Here's how the part is built. I have some questions about the finished solid (model axes, mm). Face numbers are marked on the shaded views. A direction names the side the tool comes from. Give positions to 0.01 mm unless a question says otherwise; leave off trailing zeros. Loops run counter-clockwise (first coordinate to the right, second up) from the corner with the lowest first, then second, coordinate; pieces in that order, holes last.
Q1. I'm going to push flat-ended pins straight in: P1, Ø3, axis at x = -12, z = 16.5, coming from the +Y side; P2, Ø2, axis at x = -15, z = 17.5, coming from the -Y side; P3, Ø3, axis at x = -0.5, z = 9, coming from the +Y side; P4, Ø1, axis at x = 6, z = 11, coming from the +Y side. Where does each tip first touch, or does it pass through?
Q2. I need wall thicknesses on probe 1 along X at (y, z) = (-12.5, 17.75); probe 2 along X at (y, z) = (-7.5, 9.5); probe 3 along X at (y, z) = (-13, 8). Which ranges of each line are inside material? Lowest first, please.
Q3. Thinking about a two-plate mould opening in Z: for the marked faces 4, 5 and 6, which applies, pulls with the +Z half, pulls with the -Z half, needs draft (parallel to the pull), parting line crosses it, or undercut?
Q4. Suppose I cut it at B-B (x = -16). List the corners of the cut face in (y, z) for me.
Q5. Suppose I cut it at A-A (y = -7.5). List the corners of the cut face in (x, z) for me, and give its area (3 significant figures).
Q6. Suppose I cut it at C-C (y = -13.25). List the corners of the cut face in (x, z) for me.
Q7. Suppose I cut it at D-D (z = 13.25). List the corners of the cut face in (x, y) for me, and give its area (3 significant figures).
Q8. For the marked faces 1, 2 and 3, which set-ups out of +Z, -Z, +X, -X, +Y, -Y let a thin tool reach every point of the face, with its end or its side?
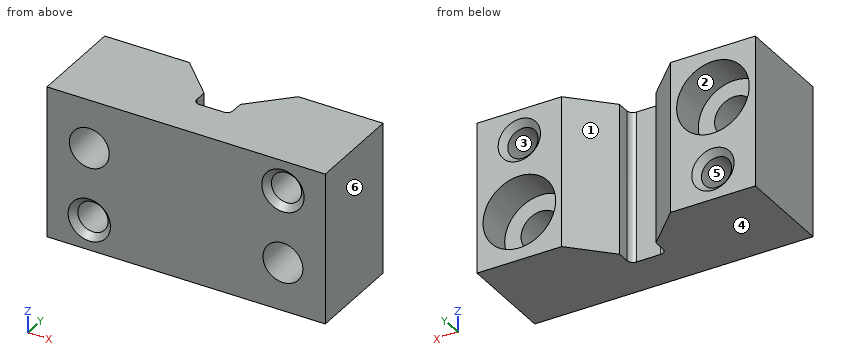
```python
from build123d import *

# Parameters (mm, degrees)
SKETCH1_W          = 46
SKETCH1_H          = 16
BOSS_EXTRUDE_DEPTH = 25
CUT_EXTRUDE1_DEPTH = 38.549966711
SKETCH4_R          = 3.3
SKETCH4_R_2        = 2.5
CUT_EXTRUDE4_DEPTH = 38.549966711
FILLET1_R          = 1
FILLET2_R          = 1
SKETCH5_R          = 6
CUT_EXTRUDE5_DEPTH = 6
CHAMFER1_SIZE      = 1
CHAMFER2_SIZE      = 1
CHAMFER3_SIZE      = 1
CHAMFER4_SIZE      = 1


with BuildPart() as part:
    # Sketch1 → Boss-Extrude (new body)
    with BuildSketch(Plane.XY):
        with Locations((0, -8)):
            Rectangle(SKETCH1_W, SKETCH1_H)
    extrude(amount=BOSS_EXTRUDE_DEPTH)

    # Sketch2 → Cut-Extrude1 (cut, through all)
    with BuildSketch(Plane.XY.offset(25)):
        Polygon((-3, -9), (3, -9), (3, -6), (9, 0), (-9, 0), (-3, -6), align=None)
    extrude(amount=-CUT_EXTRUDE1_DEPTH, mode=Mode.SUBTRACT)

    # Sketch4 → Cut-Extrude4 (cut, through all)
    with BuildSketch(Plane(origin=(0, 0, 0), x_dir=(-1, 0, 0), z_dir=(0, 1, 0))):
        with Locations(Location((16, 17, 0), (0, 0, 90))):
            Circle(SKETCH4_R)
        with Locations(Location((16, 5, 0), (0, 0, 90))):
            Circle(SKETCH4_R_2)
        with Locations(Location((-16, 20, 0), (0, 0, 90))):
            Circle(SKETCH4_R_2)
        with Locations(Location((-16, 8, 0), (0, 0, 90))):
            Circle(SKETCH4_R)
    extrude(amount=-CUT_EXTRUDE4_DEPTH, mode=Mode.SUBTRACT)

    # Fillet1
    fillet1_edges = [part.edges().sort_by_distance(p)[0] for p in [
        (-3, -9, 12.5),
    ]]
    fillet(fillet1_edges, radius=FILLET1_R)

    # Fillet2
    fillet2_edges = [part.edges().sort_by_distance(p)[0] for p in [
        (3, -9, 12.5),
    ]]
    fillet(fillet2_edges, radius=FILLET2_R)

    # Sketch5 → Cut-Extrude5 (cut)
    with BuildSketch(Plane(origin=(0, 0, 0), x_dir=(-1, 0, 0), z_dir=(0, 1, 0))):
        with Locations(Location((16, 17, 0), (0, 0, 90))):
            Circle(SKETCH5_R)
        with Locations(Location((-16, 8, 0), (0, 0, 90))):
            Circle(SKETCH5_R)
    extrude(amount=-CUT_EXTRUDE5_DEPTH, mode=Mode.SUBTRACT)

    # Chamfer1
    chamfer1_edges = [part.edges().sort_by_distance(p)[0] for p in [
        (16, 0, 17.5),
    ]]
    chamfer(chamfer1_edges, length=CHAMFER1_SIZE)

    # Chamfer2
    chamfer2_edges = [part.edges().sort_by_distance(p)[0] for p in [
        (-16, 0, 2.5),
    ]]
    chamfer(chamfer2_edges, length=CHAMFER2_SIZE)

    # Chamfer3
    chamfer3_edges = [part.edges().sort_by_distance(p)[0] for p in [
        (16, -16, 17.5),
    ]]
    chamfer(chamfer3_edges, length=CHAMFER3_SIZE)

    # Chamfer4
    chamfer4_edges = [part.edges().sort_by_distance(p)[0] for p in [
        (-16, -16, 2.5),
    ]]
    chamfer(chamfer4_edges, length=CHAMFER4_SIZE)


solid = part.part
```
Solutions:
1. P1: stops at y = -6
1. P2: passes through
1. P3: stops at y = -9
1. P4: stops at y = -2.5
2. probe 1: x = -23 to -19.21, -12.79 to 14.91, 17.09 to 23
2. probe 2: x = -23 to -3, 3 to 13.06, 18.94 to 23
2. probe 3: x = -23 to 12.7, 19.3 to 23
3. face 4: pulls with the -Z half
3. face 5: undercut
3. face 6: needs draft
4. outline: (-16, 0) - (0, 0) - (0, 1.5) - (-1, 2.5) - (-15, 2.5) - (-16, 1.5) - close; (-16, 8.5) - (-15, 7.5) - (-1, 7.5) - (0, 8.5) - (0, 11) - (-6, 11) - (-6, 13.7) - (-16, 13.7) - close; (-16, 20.3) - (-6, 20.3) - (-6, 23) - (0, 23) - (0, 25) - (-16, 25) - close
5. outline: (-23, 0) - (-3, 0) - (-3, 25) - (-23, 25) - close; (3, 0) - (23, 0) - (23, 25) - (3, 25) - close; hole circle Ø6.6 at (-16, 17); hole circle Ø5 at (-16, 5); hole circle Ø6.6 at (16, 8); hole circle Ø5 at (16, 20)
5. area: 892 mm2
6. outline: (-23, 0) - (23, 0) - (23, 25) - (-23, 25) - close; hole circle Ø6.6 at (-16, 17); hole circle Ø5 at (-16, 5); hole circle Ø6.6 at (16, 8); hole circle Ø5 at (16, 20)
7. outline: (-23, -16) - (23, -16) - (23, 0) - (18.9, 0) - (18.9, -6) - (13.1, -6) - (13.1, 0) - (9, 0) - (3, -6) - (3, -8) arc R1 cw to (2, -9) - (-2, -9) arc R1 cw to (-3, -8) - (-3, -6) - (-9, 0) - (-11.32, 0) - (-11.32, -6) - (-20.68, -6) - (-20.68, 0) - (-23, 0) - close
7. area: 555 mm2
8. face 1: +Z, -Z, +Y
8. face 2: +Y
8. face 3: +Y, -Y
